Check sheet for the modelled part. Datum: model origin and axes. Units: mm. A direction names the side the tool comes from. Round coordinates to 2 decimals unless told otherwise and drop trailing zeros. Write each loop counter-clockwise with the first axis right and the second up, starting at its lowest first coordinate (ties: lowest second). Pieces come first, ordered by that corner, then holes. Notation, with made-up numbers: (58, 2) - (92, 2) arc R14 ccw to (92, 21) - close; hole circle Ø4 at (52, 39.25). An arc over 180 degrees is marked (long way). Answer as a JSON object with one key per item and string values. Group by question number.
Item 1: Sectioned sample at B-B on x = -49.5. Record the boundary of the cut face in (y, z), plus the area to 3 significant figures.
Item 2: Set-up check for faces 1 (the flat face through (60, -57, 7)), 2 (the flat face through (-60, -57, 7)), 3 (the flat face through (-1, 234, 7)), 4 (the flat face through (33, -238, 71)), 5 (the flat face through (-6, -45, 60)): record each of +Z, -Z, +X, -X, +Y, -Y from which the full face is reachable in a straight line by a thin tool's end or side.
Item 3: Thickness scan on line 1 (X direction, y = -216, z = 8); line 2 (X direction, y = -246, z = 22); line 3 (Y direction, x = 30, z = 6). Record the ranges inside material, lowest first.
Item 4: Sectioned sample at A-A on z = 59. Record the boundary of the cut face in (x, y), plus the area to 3 significant figures.
Item 5: Gauge pin test, flat ends, axial feed: P1, Ø8.5, axis at x = -33, z = 122, coming from the -Y side; P2, Ø7.5, axis at x = 33, z = 22, coming from the +Y side; P3, Ø4, axis at x = 30, y = -66, coming from the +Z side; P4, Ø2.5, axis at x = 30, y = 34, coming from the +Z side. Record the tip position at first contact, or that the pin passes through.
```python
from build123d import *

# Parameters (mm, degrees)
SKETCH1_W                = 120
SKETCH1_H                = 500
BOSS_EXTRUDE1_DEPTH      = 12
SKETCH2_W                = 120
SKETCH2_H                = 12
BOSS_EXTRUDE2_DEPTH      = 120
BOSS_EXTRUDE3_DEPTH      = 6
M6_CLEARANCE_HOLE1_D     = 6.6
M6_CLEARANCE_HOLE1_DEPTH = 15
M6_CLEARANCE_HOLE1_TIP   = 1.982840043
M6_CLEARANCE_HOLE2_D     = 6.6
M6_CLEARANCE_HOLE2_DEPTH = 15
M6_CLEARANCE_HOLE2_TIP   = 1.982840043
M4_TAPPED_HOLE1_D        = 3.3
CUT_EXTRUDE1_DEPTH       = 308.122125546
CUT_EXTRUDE1_DEPTH_BACK  = 308.122125546
SKETCH10_W               = 7
SKETCH10_H               = 31.8


with BuildPart() as part:
    # Sketch1 → Boss-Extrude1 (new body)
    with BuildSketch(Plane.XY):
        Rectangle(SKETCH1_W, SKETCH1_H)
    extrude(amount=BOSS_EXTRUDE1_DEPTH)

    # Sketch2 → Boss-Extrude2 (add)
    with BuildSketch(Plane.XY.offset(12)):
        with Locations((0, -244)):
            Rectangle(SKETCH2_W, SKETCH2_H)
    extrude(amount=BOSS_EXTRUDE2_DEPTH)

    # Sketch3 → Boss-Extrude3 (add, symmetric)
    with BuildSketch(Plane(origin=(0, 0, 0), x_dir=(0, 0, -1), z_dir=(1, 0, 0))):
        Polygon((-12, 250), (-32, 250), (-132, -218), (-132, -238), (-12, -238), align=None)
    extrude(amount=BOSS_EXTRUDE3_DEPTH, both=True)

    # M6 Clearance Hole1
    with Locations(Plane(origin=(0, -238, 0), x_dir=(1, 0, 0), z_dir=(0, 1, 0))):
        with Locations((33, -122), (33, -22)):
            Hole(M6_CLEARANCE_HOLE1_D / 2, depth=M6_CLEARANCE_HOLE1_DEPTH)
            with Locations((0, 0, -(M6_CLEARANCE_HOLE1_DEPTH + M6_CLEARANCE_HOLE1_TIP / 2))):  # 118° drill point
                Cone(0, M6_CLEARANCE_HOLE1_D / 2, M6_CLEARANCE_HOLE1_TIP, mode=Mode.SUBTRACT)

    # M6 Clearance Hole2
    with Locations(Plane(origin=(0, -238, 0), x_dir=(1, 0, 0), z_dir=(0, 1, 0))):
        with Locations((-33, -122), (-33, -22)):
            Hole(M6_CLEARANCE_HOLE2_D / 2, depth=M6_CLEARANCE_HOLE2_DEPTH)
            with Locations((0, 0, -(M6_CLEARANCE_HOLE2_DEPTH + M6_CLEARANCE_HOLE2_TIP / 2))):  # 118° drill point
                Cone(0, M6_CLEARANCE_HOLE2_D / 2, M6_CLEARANCE_HOLE2_TIP, mode=Mode.SUBTRACT)

    # M4 Tapped Hole1 (through all)
    with Locations(Plane(origin=(0, 0, 0), x_dir=(-1, 0, 0), z_dir=(0, 0, -1))):
        with Locations((-30, 34), (-30, 134), (-30, -66), (-30, -166), (-30, -216), (30, -216), (30, -166), (30, -66), (30, 34), (30, 134)):
            Hole(M4_TAPPED_HOLE1_D / 2)

    # Sketch10 → Cut-Extrude1 (cut, two sides: drawn at the far end of the back side and taken through both)
    with BuildSketch(Plane(origin=(60, 0, 0), x_dir=(0, 0, -1), z_dir=(1, 0, 0)).offset(-CUT_EXTRUDE1_DEPTH_BACK)):
        with Locations((-3.5, 234.1)):
            Rectangle(SKETCH10_W, SKETCH10_H)
    extrude(amount=CUT_EXTRUDE1_DEPTH + CUT_EXTRUDE1_DEPTH_BACK, mode=Mode.SUBTRACT)


solid = part.part
```
Completed:
{
 "1": {"outline": "(-250, 0) - (218.2, 0) - (218.2, 7) - (250, 7) - (250, 12) - (-238, 12) - (-238, 132) - (-250, 132) - close", "area": "7,220 mm²"},
 "2": {"face 1": "+Z, -Z, +X, +Y, -Y", "face 2": "+Z, -Z, -X, +Y, -Y", "face 3": "-Z, +X, -X, +Y", "face 4": "+Z, +X, +Y", "face 5": "+Z, -X, +Y"},
 "3": {"line 1": "-60 to -31.65, -28.35 to 28.35, 31.65 to 60", "line 2": "-60 to -36.3, -29.7 to 29.7, 36.3 to 60", "line 3": "-250 to -217.65, -214.35 to -167.65, -164.35 to -67.65, -64.35 to 32.35, 35.65 to 132.35, 135.65 to 218.2"},
 "4": {"outline": "(-60, -250) - (60, -250) - (60, -238) - (6, -238) - (6, 123.64) - (-6, 123.64) - (-6, -238) - (-60, -238) - close", "area": "5,780 mm²"},
 "5": {"P1": "y = -250", "P2": "y = -238", "P3": "z = 12", "P4": "through"}
}
